Read the model definition and answer for the solid it produces. Units are mm, in the model's axes. A direction names the side the tool comes from. Coordinates: 2 decimals unless noted, no trailing zeros. Order: outer loops, then holes, each group sorted by start corner. A loop starts at its lowest first (then second) coordinate and runs counter-clockwise, first axis right, second up.
from build123d import *

# Parameters (mm, degrees)
BOSS_EXTRUDE1_DEPTH = 2
BOSS_EXTRUDE2_DEPTH = 661
BOSS_EXTRUDE3_DEPTH = 2


with BuildPart() as part:
    # Sketch1 → Boss-Extrude1 (new body)
    with BuildSketch(Plane(origin=(0, 0, 0), x_dir=(0, 0, -1), z_dir=(1, 0, 0))):
        Polygon((0, 0), (-20, 0), (-16.414240878, -29.78493464), (1.929767975, -16.029524307), align=None)
    extrude(amount=BOSS_EXTRUDE1_DEPTH)

    # Sketch2 → Boss-Extrude2 (add)
    with BuildSketch(Plane.ZY):
        Polygon((0, 0), (20, 0), (19.759223301, -2), (1.773664518, -2), (0.193910267, -15.122152246), (16.690272744, -27.492089303), (16.414240878, -29.78493464), (-1.929767975, -16.029524307), align=None)
    extrude(amount=BOSS_EXTRUDE2_DEPTH)

    # Sketch3 → Boss-Extrude3 (add)
    with BuildSketch(Plane.ZY.offset(661)):
        Polygon((20, 0), (0, 0), (-1.929767975, -16.029524307), (16.414240878, -29.78493464), align=None)
    extrude(amount=BOSS_EXTRUDE3_DEPTH)


solid = part.part
Q1. Which of the six approach directions +Z, -Z, +X, -X, +Y, -Y give full straight-line access (tool end or side, diameter ignored) to faces 4 (the flat face through (-326, 0, 10)), 5 (the flat face through (-325.873, -8.469, 0.995))?
Q2. The part is cut by section B-B, the plane z = 11. Determine the outline of the cut face in (x, y), then the cut area to 3 significant figures.
Q3. Determine the mould class of faces 1 (the flat face through (-326, -2, 11)), 2 (the flat face through (-325.84, -7.9, -0.95)), 3 (the flat face through (-325.8, -22.8, 7.1)) for opening direction Y: +Y half, -Y half, draft (parallel to the pull), parting line (faces both ways), or undercut.
Q4. The part is cut by section A-A, the plane x = -323.5. Determine the outline of the cut face in (y, z).
Q5. The part is cut by section C-C, the plane y = -9. Determine the outline of the cut face in (x, z), then the cut area to 3 significant figures.
Q6. Each of these flat-tipped pins is pushed along its axis until it touches: P1, Ø4, axis at x = -252, y = -8, coming from the -Z side; P2, Ø5.5, axis at x = -171, z = 11.5, coming from the -Y side; P3, Ø5, axis at x = -591, y = -12, coming from the -Z side. Where does it stop, or does it pass through?
Q7. Straight lines are drawn through the part: L1, parallel to X at y = -9.5, z = 18.25; L2, parallel to Z at x = -376.5, y = -1; L3, parallel to Y at x = -248, z = 2. For each, find the intervals that lie inside material, in ascending order.
Computed values:
1. face 4: +Z, -Z, +X, -X, +Y
1. face 5: +Z
2. outline: (-663, -25.73) - (2, -25.73) - (2, 0) - (-663, 0) - close; hole (-661, -23.23) - (0, -23.23) - (0, -2) - (-661, -2) - close
2. area: 3,080 mm2
3. face 1: undercut
3. face 2: +Y half
3. face 3: -Y half
4. outline: (-29.78, 16.41) - (-16.03, -1.93) - (0, 0) - (0, 20) - (-2, 19.76) - (-2, 1.77) - (-15.12, 0.19) - (-27.49, 16.69) - close
5. outline: (-663, -1.08) - (2, -1.08) - (2, 18.92) - (0, 18.92) - (0, 0.93) - (-661, 0.93) - (-661, 18.92) - (-663, 18.92) - close
5. area: 1,410 mm2
6. P1: stops at z = -1.2
6. P2: stops at y = -28.16
6. P3: stops at z = -1.75
7. L1: x = -663 to -661, 0 to 2
7. L2: z = -0.12 to 19.88
7. L3: y = -18.98 to -16.48, -2 to 0
